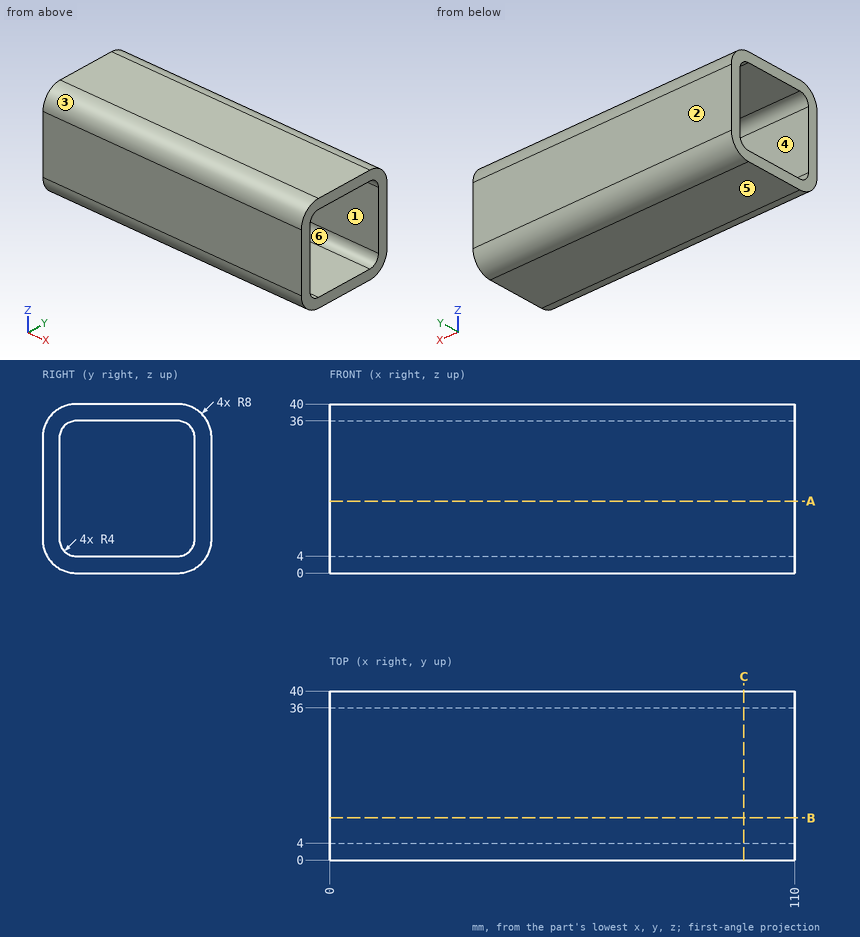
Geometry: see drawing. Coordinates: mm, zero at the bounding-box minimum. A direction names the side the tool comes from. Round coordinates to 2 decimals unless told otherwise and drop trailing zeros. Loops run counter-clockwise (first coordinate to the right, second up) from the corner with the lowest first, then second, coordinate; pieces in that order, holes last. Notation, with made-up numbers: M 12,48 L 45,48 A17 cw 45,68 Z; hole C -6,76 d2. An arc over 180 degrees is marked long. Use a Markdown table: item, result. Add a question column.
1. Set-up query: the marked faces 1 and 2. Return all of +Z, -Z, +X, -X, +Y, -Y with unobstructed straight access to the full face (end or side cutting, diameter ignored); none if empty.
2. Ray query, line 1 along Y through (x, z) = (30.5, 22); line 2 along Z through (x, y) = (33, 6.5). Return the intervals inside material, ascending. Write a range as [from, to].
3. Cut plane A-A, the plane z = 17. Output: boundary loops of the cut face in (x, y), and give its area (3 significant figures).
4. Pull-direction query (Z, two-part tool) for the marked faces 3, 4, 5 and 6; classes: +Z half, -Z half, draft (parallel to the pull), parting line (faces both ways), or undercut.
5. Contact query for a flat-ended pin moving along its axis: pin 1 (3 mm diameter, centred on x = 68.5, y = 34.5, fed in from +Z). Output: stop coordinate, or through.
6. Cut plane C-C, the plane x = 98. Output: boundary loops of the cut face in (y, z).
Solution:
| question | item | result |
|---|---|---|
| 1 | face 1 | +X, -X |
| 1 | face 2 | +Z, -Z, +X, -X, +Y |
| 2 | line 1 | y = [0, 4], [36, 40] |
| 2 | line 2 | z = [0.14, 4.29], [35.71, 39.86] |
| 3 | outline | M 0,0 L 110,0 L 110,4 L 0,4 Z; M 0,36 L 110,36 L 110,40 L 0,40 Z |
| 3 | area | 880 mm2 |
| 4 | face 3 | +Z half |
| 4 | face 4 | undercut |
| 4 | face 5 | -Z half |
| 4 | face 6 | undercut |
| 5 | pin 1 | stops at z = 39.94 |
| 6 | outline | M 0,8 A8 ccw 8,0 L 32,0 A8 ccw 40,8 L 40,32 A8 ccw 32,40 L 8,40 A8 ccw 0,32 Z; hole M 4,8 A4 ccw 8,4 L 32,4 A4 ccw 36,8 L 36,32 A4 ccw 32,36 L 8,36 A4 ccw 4,32 Z |
